```python
from build123d import *

# Parameters (mm, degrees)
SKETCH1_W            = 100
SKETCH1_H            = 300
BOSS_EXTRUDE1_DEPTH  = 6
M6_TAPPED_HOLE1_D    = 5
LPATTERN1_COUNT      = 3
LPATTERN1_PITCH      = 70
LPATTERN1_COUNT_DIR2 = 2
LPATTERN1_PITCH_DIR2 = 70
LPATTERN2_COUNT      = 3
LPATTERN2_PITCH      = 70
LPATTERN2_COPY_1_D   = 5
LPATTERN2_COPY_2_D   = 5
LPATTERN2_COPY_3_D   = 5
LPATTERN2_COPY_4_D   = 5
LPATTERN2_COPY_5_D   = 5
LPATTERN2_COPY_6_D   = 5
LPATTERN2_COPY_7_D   = 5
LPATTERN2_COPY_8_D   = 5
LPATTERN2_COPY_9_D   = 5
LPATTERN2_COPY_10_D  = 5


with BuildPart() as part:
    # Sketch1 → Boss-Extrude1 (new body)
    with BuildSketch(Plane.XY):
        Rectangle(SKETCH1_W, SKETCH1_H)
    extrude(amount=BOSS_EXTRUDE1_DEPTH)

    # M6 Tapped Hole1 (through all)
    with Locations(Plane.XY.offset(6)):
        with Locations((-35, 0)):
            m6_tapped_hole1 = Hole(M6_TAPPED_HOLE1_D / 2)

    # LPattern1: M6 Tapped Hole1 3 × 2
    with Locations(*[(j * LPATTERN1_PITCH_DIR2, -i * LPATTERN1_PITCH, 0) for i in range(LPATTERN1_COUNT) for j in range(LPATTERN1_COUNT_DIR2) if (i, j) != (0, 0)]):
        add(m6_tapped_hole1, mode=Mode.SUBTRACT)

    # LPattern2: M6 Tapped Hole1 ×3
    with Locations(*[(0, i * LPATTERN2_PITCH, 0) for i in range(1, LPATTERN2_COUNT)]):
        add(m6_tapped_hole1, mode=Mode.SUBTRACT)

    # LPattern2 copy 1 (through all)
    with Locations(Plane(origin=(70, 70, 6), x_dir=(1, 0, 0), z_dir=(0, 0, 1))):
        with Locations((-35, 0)):
            Hole(LPATTERN2_COPY_1_D / 2)

    # LPattern2 copy 2 (through all)
    with Locations(Plane(origin=(70, 140, 6), x_dir=(1, 0, 0), z_dir=(0, 0, 1))):
        with Locations((-35, 0)):
            Hole(LPATTERN2_COPY_2_D / 2)

    # LPattern2 copy 3 (through all)
    with Locations(Plane.XY.offset(6)):
        with Locations((-35, 0)):
            Hole(LPATTERN2_COPY_3_D / 2)

    # LPattern2 copy 4 (through all)
    with Locations(Plane(origin=(0, 70, 6), x_dir=(1, 0, 0), z_dir=(0, 0, 1))):
        with Locations((-35, 0)):
            Hole(LPATTERN2_COPY_4_D / 2)

    # LPattern2 copy 5 (through all)
    with Locations(Plane(origin=(70, 0, 6), x_dir=(1, 0, 0), z_dir=(0, 0, 1))):
        with Locations((-35, 0)):
            Hole(LPATTERN2_COPY_5_D / 2)

    # LPattern2 copy 6 (through all)
    with Locations(Plane(origin=(70, 70, 6), x_dir=(1, 0, 0), z_dir=(0, 0, 1))):
        with Locations((-35, 0)):
            Hole(LPATTERN2_COPY_6_D / 2)

    # LPattern2 copy 7 (through all)
    with Locations(Plane(origin=(0, -70, 6), x_dir=(1, 0, 0), z_dir=(0, 0, 1))):
        with Locations((-35, 0)):
            Hole(LPATTERN2_COPY_7_D / 2)

    # LPattern2 copy 8 (through all)
    with Locations(Plane.XY.offset(6)):
        with Locations((-35, 0)):
            Hole(LPATTERN2_COPY_8_D / 2)

    # LPattern2 copy 9 (through all)
    with Locations(Plane(origin=(70, -70, 6), x_dir=(1, 0, 0), z_dir=(0, 0, 1))):
        with Locations((-35, 0)):
            Hole(LPATTERN2_COPY_9_D / 2)

    # LPattern2 copy 10 (through all)
    with Locations(Plane(origin=(70, 0, 6), x_dir=(1, 0, 0), z_dir=(0, 0, 1))):
        with Locations((-35, 0)):
            Hole(LPATTERN2_COPY_10_D / 2)


solid = part.part
```
Could you check a few things on this model? Use its own coordinates, in mm. Give positions to 0.01 mm unless a question says otherwise; leave off trailing zeros. One line per item, written item: value. Start each with the question number.
Item 1: I'm going to push a flat-ended pin straight in: pin 1 (4 mm diameter, centred on x = -35, y = -140, fed in from +Z). Where does the tip first touch, or does it pass through?
Item 2: If we mould it in two halves opening along X, with no side actions, what happens to faces 1 (the face through (32.69, 69.04, 2.96)), 2 (the face through (-50, -2, 3)), 3 (the face through (-1, 150, 3)), 4 (the face through (33.66, 142.11, 2.96))? For each: +X half, -X half, draft (parallel to the pull), parting line (faces both ways), or undercut.
Item 3: Please list where these lines run through material, in increasing order: line 1 (X direction, y = -140, z = 2.7); line 2 (Y direction, x = -35, z = 1.35). Write a range as from..to.
Geometry says:
1. pin 1: through
2. face 1: undercut
2. face 2: -X half
2. face 3: draft
2. face 4: undercut
3. line 1: -50..-37.5, -32.5..32.5, 37.5..50
3. line 2: -150..-142.5, -137.5..-72.5, -67.5..-2.5, 2.5..67.5, 72.5..137.5, 142.5..150
